Source: CAD feature listing. Evaluate the final solid. Frame: model axes, mm. A direction names the side the tool comes from. Give positions to 0.01 mm unless a question says otherwise; leave off trailing zeros. Order: outer loops, then holes, each group sorted by start corner. A loop starts at its lowest first (then second) coordinate and runs counter-clockwise, first axis right, second up. Notation, with made-up numbers: M -37,89.5 L -30,89.5 A16 cw -30,109.5 Z; hole C 26,-33.5 d5. An arc over 180 degrees is marked long. Use CSV: the item, a comma, the result in double quotes. Start each with the question number.
Item 1: Section query A-A on x = -37.5. Return loops of the section in (y, z).
Item 2: Section query B-B on z = -5.5. Return loops of the section in (x, y), and give its area (3 significant figures).
Item 3: Pull-direction query (X, two-part tool) for faces 3 (the face through (0.93, -88.73, 0.22)), 4 (the face through (0, -11, 35)), 5 (the face through (-38.46, 0.01, -35.19)); classes: +X half, -X half, draft (parallel to the pull), parting line (faces both ways), or undercut.
Item 4: Section query C-C on y = -51.5. Return loops of the section in (x, z).
Item 5: Access query for faces 1 (the face through (-13, -41.75, 0)), 2 (the face through (-47.97, 0.01, 47.79)). Directions: +Z, -Z, +X, -X, +Y, -Y. A direction counts if a zero-diameter tool reaches every point of the face in a straight line with its end or side. Return the directions, or none.
Item 6: First-contact query: pin 1 (14 mm diameter, centred on x = 6.5, y = -54, fed in from +Z); pin 2 (11 mm diameter, centred on x = 11.5, z = -5, fed in from -Y); pin 3 (10 mm diameter, centred on x = 7, y = -22, fed in from +Z). Flat tips, straight axial feed; report the tip coordinate or a pass-through.
Item 7: Section query D-D on x = 0. Return loops of the section in (y, z), and give its area (3 significant figures).
Item 8: Ray query, probe 1 along X at (y, z) = (-0.2, 50); probe 2 along X at (y, z) = (0.15, 25); probe 3 along Y at (x, z) = (0, -6.5). Return the intervals inside material, ascending. Write a range as from..to.
from build123d import *

# Parameters (mm, degrees)
SKETCH_1_W          = 115
SKETCH_1_H          = 115
EXTRUDE_1_DEPTH     = 0.75
SKETCH_2_R          = 2.5
CUT_EXTRUDE_1_DEPTH = 82.331113358
SKETCH_3_R          = 2.5
CUT_EXTRUDE_2_DEPTH = 82.331113358
SKETCH_4_R          = 3
CUT_EXTRUDE_3_DEPTH = 82.331113358
FILLET_1_R          = 3
SKETCH_5_W          = 35
SKETCH_5_H          = 70
EXTRUDE_2_DEPTH     = 41
CHAMFER_1_SIZE      = 20
SKETCH_6_R          = 18.5
EXTRUDE_3_DEPTH     = 15.5


with BuildPart() as part:
    # 草图1 → 凸台-拉伸1 (new, symmetric)
    with BuildSketch(Plane(origin=(0, 0, 0), x_dir=(1, 0, 0), z_dir=(0, 1, 0))):
        Rectangle(SKETCH_1_W, SKETCH_1_H)
    extrude(amount=EXTRUDE_1_DEPTH, both=True)

    # 草图2 → 切除-拉伸1 (cut, through all)
    with BuildSketch(Plane(origin=(0, 0.75, 0), x_dir=(1, 0, 0), z_dir=(0, 1, 0))):
        with Locations(Location((-25, 25, 0), (0, 0, 270))):
            Circle(SKETCH_2_R)
        with Locations(Location((25, 25, 0), (0, 0, 270))):
            Circle(SKETCH_2_R)
        with Locations(Location((25, -25, 0), (0, 0, 270))):
            Circle(SKETCH_2_R)
        with Locations(Location((-25, -25, 0), (0, 0, 270))):
            Circle(SKETCH_2_R)
    extrude(amount=-CUT_EXTRUDE_1_DEPTH, mode=Mode.SUBTRACT)

    # 草图3 → 切除-拉伸2 (cut, through all)
    with BuildSketch(Plane(origin=(0, 0.75, 0), x_dir=(1, 0, 0), z_dir=(0, 1, 0))):
        with Locations(Location((-37.5, 37.5, 0), (0, 0, 270))):
            Circle(SKETCH_3_R)
        with Locations(Location((-37.5, -37.5, 0), (0, 0, 270))):
            Circle(SKETCH_3_R)
        with Locations(Location((37.5, -37.5, 0), (0, 0, 270))):
            Circle(SKETCH_3_R)
        with Locations(Location((37.5, 37.5, 0), (0, 0, 270))):
            Circle(SKETCH_3_R)
    extrude(amount=-CUT_EXTRUDE_2_DEPTH, mode=Mode.SUBTRACT)

    # 草图4 → 切除-拉伸3 (cut, through all)
    with BuildSketch(Plane(origin=(0, 0.75, 0), x_dir=(1, 0, 0), z_dir=(0, 1, 0))):
        with Locations(Location((-50, 50, 0), (0, 0, 270))):
            Circle(SKETCH_4_R)
        with Locations(Location((50, 50, 0), (0, 0, 270))):
            Circle(SKETCH_4_R)
        with Locations(Location((-50, -50, 0), (0, 0, 270))):
            Circle(SKETCH_4_R)
        with Locations(Location((50, -50, 0), (0, 0, 270))):
            Circle(SKETCH_4_R)
    extrude(amount=-CUT_EXTRUDE_3_DEPTH, mode=Mode.SUBTRACT)

    # 圆角1
    fillet_1_edges = [part.edges().sort_by_distance(p)[0] for p in [
        (-57.5, 0, -57.5),
        (57.5, 0, -57.5),
        (57.5, 0, 57.5),
        (-57.5, 0, 57.5),
    ]]
    fillet(fillet_1_edges, radius=FILLET_1_R)

    # 草图5 → 凸台-拉伸2 (add)
    with BuildSketch(Plane.XZ.offset(0.75)):
        Rectangle(SKETCH_5_W, SKETCH_5_H)
    extrude(amount=EXTRUDE_2_DEPTH)

    # 倒角1
    chamfer_1_edges = [part.edges().sort_by_distance(p)[0] for p in [
        (0, -41.75, -35),
        (0, -41.75, 35),
    ]]
    chamfer(chamfer_1_edges, length=CHAMFER_1_SIZE)

    # 草图6 → 凸台-拉伸3 (add, symmetric)
    with BuildSketch(Plane.XY):
        with BuildLine():
            Line((7.5, -41.75), (7.5, -42.978942549))
            ThreePointArc((7.5, -42.978942549), (0, -88.75), (-7.5, -42.978942549))
            Line((-7.5, -42.978942549), (-7.5, -41.75))
            Line((-7.5, -41.75), (7.5, -41.75))
        make_face()
        with Locations((0, -65.25)):
            Circle(SKETCH_6_R, mode=Mode.SUBTRACT)
    extrude(amount=EXTRUDE_3_DEPTH, both=True)


solid = part.part
Verdict:
1,outline,"M -0.75,-57.5 L 0.75,-57.5 L 0.75,-40 L -0.75,-40 Z; M -0.75,-35 L 0.75,-35 L 0.75,35 L -0.75,35 Z; M -0.75,40 L 0.75,40 L 0.75,57.5 L -0.75,57.5 Z"
2,outline,"M -57.5,-0.75 L -17.5,-0.75 L -17.5,-41.75 L -7.5,-41.75 L -7.5,-42.98 A23.5 ccw long 7.5,-42.98 L 7.5,-41.75 L 17.5,-41.75 L 17.5,-0.75 L 57.5,-0.75 L 57.5,0.75 L -57.5,0.75 Z; hole C 0,-65.25 d37"
2,area,"2,270 mm2"
3,face 3,"parting line"
3,face 4,"draft"
3,face 5,"undercut"
4,outline,"M -19.06,-15.5 L -12.38,-15.5 L -12.38,15.5 L -19.06,15.5 Z; M 12.38,-15.5 L 19.06,-15.5 L 19.06,15.5 L 12.38,15.5 Z"
5,face 1,"+Z, -Z, -X"
5,face 2,"+Y, -Y"
6,pin 1,"z = 15.5"
6,pin 2,"y = -87.97"
6,pin 3,"z = 35"
7,outline,"M -88.75,-15.5 L -83.75,-15.5 L -83.75,15.5 L -88.75,15.5 Z; M -46.75,-15.5 L -41.75,-15.5 L -41.75,-15 L -21.75,-35 L -0.75,-35 L -0.75,-57.5 L 0.75,-57.5 L 0.75,57.5 L -0.75,57.5 L -0.75,35 L -21.75,35 L -41.75,15 L -41.75,15.5 L -46.75,15.5 Z"
7,area,"2,950 mm2"
8,probe 1,"-57.5..-53, -47..47, 53..57.5"
8,probe 2,"-57.5..-27.5, -22.5..22.5, 27.5..57.5"
8,probe 3,"-88.75..-83.75, -46.75..0.75"
